Work out the finished part from the listing and answer in its coordinate system (mm). Face numbers are marked on the shaded views. Coordinates: 2 decimals unless noted, no trailing zeros. Write each loop counter-clockwise with the first axis right and the second up, starting at its lowest first coordinate (ties: lowest second). Pieces come first, ordered by that corner, then holes. Notation, with made-up numbers: (45.5, -7) - (56.5, -7) arc R22 cw to (56.5, 0) - close; hole circle Ø8 at (45, -19.5). An arc over 180 degrees is marked (long way). Answer as a JSON object with one key per item and string values. Group by question number.
from build123d import *

# Parameters (mm, degrees)
SKETCH_1_W                = 950
SKETCH_1_H                = 55
EXTRUDE_1_DEPTH           = 6
SKETCH_2_W                = 790
SKETCH_2_H                = 23
CUT_EXTRUDE_1_DEPTH       = 12
CHAMFER_1_SIZE            = 5
HOLE_WIZARD_M8_1_D        = 9
HOLE_WIZARD_1_D           = 6.6
HOLE_WIZARD_1_CBORE_D     = 11
HOLE_WIZARD_1_CBORE_DEPTH = 6.8


with BuildPart() as part:
    # 草图1 → 凸台-拉伸1 (new, symmetric)
    with BuildSketch(Plane(origin=(0, 0, 0), x_dir=(1, 0, 0), z_dir=(0, 1, 0))):
        Rectangle(SKETCH_1_W, SKETCH_1_H)
    extrude(amount=EXTRUDE_1_DEPTH, both=True)

    # 草图2 → 切除-拉伸1 (cut)
    with BuildSketch(Plane(origin=(0, 6, 0), x_dir=(1, 0, 0), z_dir=(0, 1, 0))):
        with Locations((0, 16)):
            Rectangle(SKETCH_2_W, SKETCH_2_H)
    extrude(amount=-CUT_EXTRUDE_1_DEPTH, mode=Mode.SUBTRACT)

    # 倒角1
    chamfer_1_edges = [part.edges().sort_by_distance(p)[0] for p in [
        (-395, 0, -27.5),
        (395, 0, -27.5),
        (475, 0, 27.5),
        (-475, 0, 27.5),
        (-475, 0, -27.5),
        (475, 0, -27.5),
    ]]
    chamfer(chamfer_1_edges, length=CHAMFER_1_SIZE)

    # M8 间隙孔1 (through all)
    with Locations(Plane(origin=(0, -6, 0), x_dir=(-1, 0, 0), z_dir=(0, -1, 0))):
        with Locations((462, 15), (-462, 15)):
            Hole(HOLE_WIZARD_M8_1_D / 2)

    # 打孔尺寸(%根据)内六角圆柱头螺钉的类型1 (through all)
    with Locations(Plane(origin=(0, 6, 0), x_dir=(1, 0, 0), z_dir=(0, 1, 0))):
        with Locations((55, -1.5), (0, -1.5), (-55, -1.5)):
            CounterBoreHole(HOLE_WIZARD_1_D / 2, HOLE_WIZARD_1_CBORE_D / 2, HOLE_WIZARD_1_CBORE_DEPTH)


solid = part.part
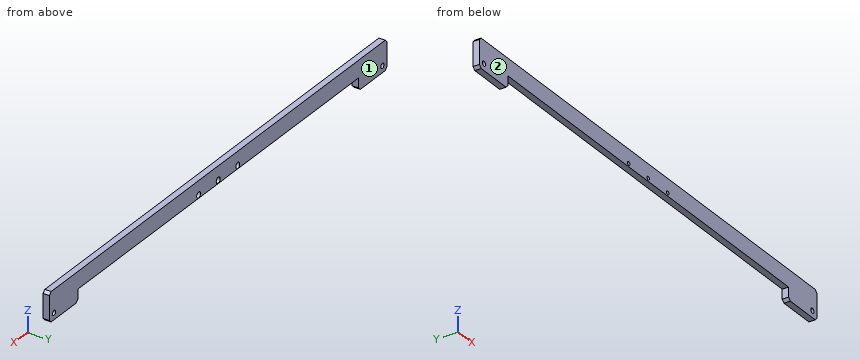
Q1. Flat-ended cylindrical pins translate along their axes: pin 1 Ø10 at (x, z) = (0, 1.5) entering from -Y; pin 2 Ø7.5 at (x, z) = (-55, 1.5) entering from +Y; pin 3 Ø2 at (x, y) = (-114.5, 4) entering from -Z; pin 4 Ø5.5 at (x, z) = (0, 2) entering from +Y. Find the tip coordinate at first contact, or state that the pin passes through.
Q2. Consider L1, parallel to X at y = -0.75, z = -14; L2, parallel to Z at x = 0, y = 0.75; L3, parallel to X at y = 1.5, z = -1.5. Determine where each line is inside the solid, lowest interval first. Write a range as from..to.
Q3. Section B-B on x = -263 is taken. Determine the outline of the cut face in (y, z), plus the area to 3 significant figures.
Q4. Section A-A on y = 3.25 is taken. Determine the outline of the cut face in (x, z), plus the area to 3 significant figures.
Q5. For a pull along Y with two mould halves and no side action, classify the marked faces 1 and 2 as +Y half, -Y half, draft (parallel to the pull), parting line (faces both ways), or undercut.
Numbers:
{
 "1": {"pin 1": "stops at y = -6", "pin 2": "stops at y = -0.8", "pin 3": "stops at z = -4.5", "pin 4": "passes through"},
 "2": {"L1": "x = -475..-466.39, -457.61..-395, 395..457.61, 466.39..475", "L2": "z = -4.5..-4, 7..27.5", "L3": "x = -475..-59.61, -50.39..-4.61, 4.61..50.39, 59.61..475"},
 "3": {"outline": "(-6, -4.5) - (6, -4.5) - (6, 27.5) - (-6, 27.5) - close", "area": "384 mm²"},
 "4": {"outline": "(-475, -22.5) - (-470, -27.5) - (-400, -27.5) - (-395, -22.5) - (-395, -4.5) - (395, -4.5) - (395, -22.5) - (400, -27.5) - (470, -27.5) - (475, -22.5) - (475, 22.5) - (470, 27.5) - (-470, 27.5) - (-475, 22.5) - close; hole circle Ø9 at (-462, -15); hole circle Ø11 at (-55, 1.5); hole circle Ø11 at (0, 1.5); hole circle Ø11 at (55, 1.5); hole circle Ø9 at (462, -15)", "area": "33,600 mm²"},
 "5": {"face 1": "+Y half", "face 2": "-Y half"}
}
